```python
from build123d import *

# Parameters (mm, degrees)
BASE_PLATE_AND_COLUMN_SKETCH_R = 5
BASE_PLATE_AND_COLUMN_SKETCH_W = 18
BASE_PLATE_AND_COLUMN_SKETCH_H = 40
BASE_PLATE_DEPTH               = 10
FRONT_PROFILE_SKETCH_R         = 4.377272593
FRONT_PROFILE_BOSS_40MM_DEPTH  = 40
UPRIGHT_COLUMN_100MM_DEPTH     = 100
COLUMN_EDGE_FILLETS_RADIUS     = 28.912605022
COLUMN_EDGE_FILLETS_LENGTH     = 10
SKETCH2_6_R                    = 4.295746386
SKETCH2_6_R_2                  = 7.787765557
SKETCH2_6_R_3                  = 2.809047726
THROUGH_CUT_A_DEPTH            = 100
SKETCH2_7_R                    = 3
THROUGH_CUT_B_DEPTH            = 100


with BuildPart() as part:
    # Base Plate and Column Sketch → Base Plate (new body)
    # profile 1 of 4: a face of its own
    with BuildSketch(Plane(origin=(0, 0, 0), x_dir=(1, 0, 0), z_dir=(0, 1, 0))):
        with BuildLine():
            Line((53, 40), (53, 0))
            Line((53, 0), (62, 0))
            ThreePointArc((62, 0), (67.656854249, 2.343145751), (70, 8))
            Line((70, 8), (70, 32))
            ThreePointArc((70, 32), (68.296857954, 36.934529351), (63.912605022, 39.768007597))
            ThreePointArc((63.912605022, 39.768007597), (62.963311793, 39.941790125), (62, 40))
            Line((62, 40), (53, 40))
        make_face()
        with Locations(Location((62, 10, 0), (0, 0, 270))):
            Circle(BASE_PLATE_AND_COLUMN_SKETCH_R, mode=Mode.SUBTRACT)
        with Locations(Location((62, 30, 0), (0, 0, 270))):
            Circle(BASE_PLATE_AND_COLUMN_SKETCH_R, mode=Mode.SUBTRACT)
    # profile 2 of 4: a face of its own
    with BuildSketch(Plane(origin=(0, 0, 0), x_dir=(1, 0, 0), z_dir=(0, 1, 0))):
        with BuildLine():
            ThreePointArc((0, 8), (2.343145751, 2.343145751), (8, 0))
            Line((8, 0), (17, 0))
            Line((17, 0), (17, 40))
            Line((17, 40), (8, 40))
            ThreePointArc((8, 40), (7.036688207, 39.941790125), (6.087394978, 39.768007597))
            ThreePointArc((6.087394978, 39.768007597), (1.703142046, 36.934529351), (0, 32))
            Line((0, 32), (0, 8))
        make_face()
        with Locations(Location((8, 10, 0), (0, 0, 270))):
            Circle(BASE_PLATE_AND_COLUMN_SKETCH_R, mode=Mode.SUBTRACT)
        with Locations(Location((8, 30, 0), (0, 0, 270))):
            Circle(BASE_PLATE_AND_COLUMN_SKETCH_R, mode=Mode.SUBTRACT)
    # profile 3 of 4: a face of its own
    with BuildSketch(Plane(origin=(0, 0, 0), x_dir=(1, 0, 0), z_dir=(0, 1, 0))):
        with Locations((26, 20)):
            Rectangle(BASE_PLATE_AND_COLUMN_SKETCH_W, BASE_PLATE_AND_COLUMN_SKETCH_H)
    # profile 4 of 4: a face of its own
    with BuildSketch(Plane(origin=(0, 0, 0), x_dir=(1, 0, 0), z_dir=(0, 1, 0))):
        with Locations((44, 20)):
            Rectangle(BASE_PLATE_AND_COLUMN_SKETCH_W, BASE_PLATE_AND_COLUMN_SKETCH_H)
    extrude(amount=BASE_PLATE_DEPTH)

    # Front Profile Sketch → Front Profile Boss 40mm (add)
    with BuildSketch(Plane.XY):
        with BuildLine():
            ThreePointArc((26.016312226, 15.260465273), (23.087140841, 11.445754131), (18.5, 10))
            Line((18.5, 10), (51.5, 10))
            ThreePointArc((51.5, 10), (46.912859159, 11.445754131), (43.983687774, 15.260465273))
            ThreePointArc((43.983687774, 15.260465273), (43.897725001, 16.317658687), (44.364453302, 17.270135567))
            ThreePointArc((44.364453302, 17.270135567), (46.68986027, 21.123183149), (47.5, 25.550051892))
            Line((47.5, 25.550051892), (47.5, 51.048166153))
            ThreePointArc((47.5, 51.048166153), (52.970478526, 62.969513929), (48.898595899, 75.438051934))
            Line((48.898595899, 75.438051934), (39.895129219, 86.378336678))
            ThreePointArc((39.895129219, 86.378336678), (34.372816044, 88.537489), (29.361733435, 85.367799323))
            Line((29.361733435, 85.367799323), (21.162337749, 75.511694203))
            ThreePointArc((21.162337749, 75.511694203), (17.026848791, 63.017230636), (22.5, 51.048166153))
            Line((22.5, 51.048166153), (22.5, 25.550051892))
            ThreePointArc((22.5, 25.550051892), (23.31013973, 21.123183149), (25.635546698, 17.270135567))
            ThreePointArc((25.635546698, 17.270135567), (26.102274999, 16.317658687), (26.016312226, 15.260465273))
        make_face()
        with Locations((35, 46)):
            Circle(FRONT_PROFILE_SKETCH_R, mode=Mode.SUBTRACT)
        with BuildLine():
            Line((34.943116214, 73.99983821), (34.943118802, 74.000202219))
            ThreePointArc((34.943118802, 74.000202219), (34.971559221, 74.000050555), (35, 74))
            ThreePointArc((35, 74), (42.071067812, 71.071067812), (45, 64))
            ThreePointArc((45, 64), (27.949072326, 56.908849252), (34.943116214, 73.99983821))
        make_face(mode=Mode.SUBTRACT)
        with BuildLine():
            ThreePointArc((38, 82), (37.113765438, 79.871151562), (34.978669551, 79.000075832))
            ThreePointArc((34.978669551, 79.000075832), (32.000018958, 82.010665292), (35, 85))
            ThreePointArc((35, 85), (37.121320344, 84.121320344), (38, 82))
        make_face(mode=Mode.SUBTRACT)
    extrude(amount=-FRONT_PROFILE_BOSS_40MM_DEPTH)

    # Sketch1_3 → Upright Column 100mm (add)
    with BuildSketch(Plane(origin=(0, 0, 0), x_dir=(1, 0, 0), z_dir=(0, 1, 0))):
        with BuildLine():
            Line((8, 40), (17, 40))
            Line((17, 40), (53, 40))
            Line((53, 40), (62, 40))
            ThreePointArc((62, 40), (62.963311793, 39.941790125), (63.912605022, 39.768007597))
            Line((63.912605022, 39.768007597), (63.912605022, 49.768007597))
            Line((63.912605022, 49.768007597), (6.087394978, 49.768007597))
            Line((6.087394978, 49.768007597), (6.087394978, 39.768007597))
            ThreePointArc((6.087394978, 39.768007597), (7.036688207, 39.941790125), (8, 40))
        make_face()
    extrude(amount=UPRIGHT_COLUMN_100MM_DEPTH)

    # Column Edge Fillets: full round fillet: the end face becomes a half cylinder, R = half its width
    column_edge_fillets_face = Plane((35, 100, -44.768007597), x_dir=(0, 0, 1), z_dir=(0, 1, 0))  # on the end face: x along it, z out of the body
    column_edge_fillets_slab = column_edge_fillets_face.offset(-COLUMN_EDGE_FILLETS_RADIUS / 2) * Box(COLUMN_EDGE_FILLETS_LENGTH, 2 * COLUMN_EDGE_FILLETS_RADIUS, COLUMN_EDGE_FILLETS_RADIUS, mode=Mode.PRIVATE)  # the body's end, R deep
    column_edge_fillets_round = Plane((35, 71.087394978, -44.768007597), x_dir=(0, 1, 0), z_dir=(0, 0, 1)) * Cylinder(COLUMN_EDGE_FILLETS_RADIUS, COLUMN_EDGE_FILLETS_LENGTH, mode=Mode.PRIVATE)  # its axis R under the face
    add(column_edge_fillets_slab - column_edge_fillets_round, mode=Mode.SUBTRACT)

    # Sketch2_6 → Through Cut A (cut)
    with BuildSketch(Plane.XY):
        with Locations((35, 46)):
            Circle(SKETCH2_6_R)
        with Locations((35, 64)):
            Circle(SKETCH2_6_R_2)
        with Locations((35, 82)):
            Circle(SKETCH2_6_R_3)
    extrude(amount=-THROUGH_CUT_A_DEPTH, mode=Mode.SUBTRACT)

    # Sketch2_7 → Through Cut B (cut)
    with BuildSketch(Plane.XY):
        with Locations((59, 64.824567346)):
            Circle(SKETCH2_7_R)
        with Locations((59, 32.824567346)):
            Circle(SKETCH2_7_R)
        with Locations(Location((11, 34.383225645, 0), (0, 0, 180))):
            Circle(SKETCH2_7_R)
        with Locations(Location((11, 66.383225645, 0), (0, 0, 180))):
            Circle(SKETCH2_7_R)
    extrude(amount=-THROUGH_CUT_B_DEPTH, mode=Mode.SUBTRACT)


solid = part.part
```
CAD build for the part. Positions are in the model's coordinates, mm. A direction names the side the tool comes from. Give positions to 0.01 mm unless a question says otherwise; leave off trailing zeros. Write each loop counter-clockwise with the first axis right and the second up, starting at its lowest first coordinate (ties: lowest second). Pieces come first, ordered by that corner, then holes. Notation, with made-up numbers: (20, 17) -> (38, 17) arc R18 cw to (38, 23) -> close; hole circle Ø11 at (43.25, 41.5). An arc over 180 degrees is marked (long way). Write each question's results on one line, items separated by ' | '.
1. Cut at B-B, the plane y = 28. Write the cut outline in (x, z), then the cut area to 3 significant figures.
Geometry check:
outline: (6.09, -49.77) -> (63.91, -49.77) -> (63.91, -39.77) arc R8 cw to (62, -40) -> (47.5, -40) -> (47.5, 0) -> (22.5, 0) -> (22.5, -40) -> (8, -40) arc R8 cw to (6.09, -39.77) -> close | area: 1,570 mm²
2. Cut at A-A, the plane z = -16.5. Give the number of separate pieces and of enclosed holes in the cut face, then the cut area to 3 significant figures.
Geometry check:
separate pieces: 1 | enclosed holes: 3 | area: 2,300 mm²
3. Cut at D-D, the plane x = 11. Write the cut outline in (y, z).
Geometry check:
outline: (0, -49.77) -> (31.38, -49.77) -> (31.38, -40) -> (10, -40) -> (10, -34) -> (0, -34) -> close; (0, -26) -> (10, -26) -> (10, -14) -> (0, -14) -> close; (0, -6) -> (10, -6) -> (10, 0) -> (0, 0) -> close; (37.38, -49.77) -> (63.38, -49.77) -> (63.38, -40) -> (37.38, -40) -> close; (69.38, -49.77) -> (87.21, -49.77) -> (87.21, -40) -> (69.38, -40) -> close
4. Drop flat-ended pins along their axis: P1, Ø20.5, axis at y = 32, z = -17.5, coming from the -X side; P2, Ø10, axis at x = 34, y = 60.5, coming from the +Z side; P3, Ø2, axis at y = 63, z = -38.5, coming from the -X side. Give the stop position or say it passes through.
Geometry check:
P1: x = 22.5 | P2: z = -40 | P3: x = 17
5. Wall check: probe 1 along Y at (x, z) = (35, -46.75); probe 2 along Y at (x, z) = (35, -3); probe 3 along X at (y, z) = (64, -9). Give the ranges that are in metal, low to high. Write a range as [from, to].
Geometry check:
probe 1: [0, 41.7], [50.3, 56.21], [71.79, 79.19], [84.81, 100] | probe 2: [0, 41.62], [50.38, 54], [74, 79], [85, 88.57] | probe 3: [17, 25], [45, 53]
6. Two-plate mould, pull along Z, no slides. Class faces 4 (the flat face through (35, 34, 0)), 5 (the cylindrical face through (17.018, 63.206, -19.72)), 6 (the cylindrical face through (8, 5, -35)): pulls with the +Z half, pulls with the -Z half, needs draft (parallel to the pull), parting line crosses it, or undercut.
Geometry check:
face 4: pulls with the +Z half | face 5: needs draft | face 6: undercut
7. Which spindle directions (+Z, -Z, +X, -X, +Y, -Y) get a long thin tool onto all of the face, cutting with end or side? Do faces 1 (the cylindrical face through (23.29, 21.18, -19.72)), 2 (the flat face through (70, 5, -20)), 3 (the cylindrical face through (43.895, 16.303, -19.72)). Say none if no direction does.
Geometry check:
face 1: +Z, -X | face 2: +Z, -Z, +X, +Y, -Y | face 3: +Z, +X
